from build123d import *

# Parameters (mm, degrees)
BOSS_EXTRUDE1_DEPTH = 35
SKETCH2_W           = 34.392896322
SKETCH2_H           = 15.037586703
CUT_EXTRUDE1_DEPTH  = 14
SKETCH3_R           = 2.25
CUT_EXTRUDE2_DEPTH  = 19


with BuildPart() as part:
    # Sketch1 → Boss-Extrude1 (new body)
    with BuildSketch(Plane.XY):
        with BuildLine():
            Line((-24, 0), (-14.5, 0))
            ThreePointArc((-14.5, 0), (-12.732233047, 0.732233047), (-12, 2.5))
            Line((-12, 2.5), (-12, 15.5))
            ThreePointArc((-12, 15.5), (-11.267766953, 17.267766953), (-9.5, 18))
            Line((-9.5, 18), (9.5, 18))
            ThreePointArc((9.5, 18), (11.267766953, 17.267766953), (12, 15.5))
            Line((12, 15.5), (12, 2.5))
            ThreePointArc((12, 2.5), (12.732233047, 0.732233047), (14.5, 0))
            Line((14.5, 0), (24, 0))
            Line((24, 0), (24, 2))
            Line((24, 2), (16.5, 2))
            ThreePointArc((16.5, 2), (14.732233047, 2.732233047), (14, 4.5))
            Line((14, 4.5), (14, 17.5))
            ThreePointArc((14, 17.5), (13.267766953, 19.267766953), (11.5, 20))
            Line((11.5, 20), (-11.5, 20))
            ThreePointArc((-11.5, 20), (-13.267766953, 19.267766953), (-14, 17.5))
            Line((-14, 17.5), (-14, 4.5))
            ThreePointArc((-14, 4.5), (-14.732233047, 2.732233047), (-16.5, 2))
            Line((-16.5, 2), (-24, 2))
            Line((-24, 2), (-24, 0))
        make_face()
    extrude(amount=BOSS_EXTRUDE1_DEPTH)

    # Sketch2 → Cut-Extrude1 (cut)
    with BuildSketch(Plane.XY.offset(35)):
        with Locations((0, 21.518793352)):
            Rectangle(SKETCH2_W, SKETCH2_H)
    extrude(amount=-CUT_EXTRUDE1_DEPTH, mode=Mode.SUBTRACT)

    # Sketch3 → Cut-Extrude2 (cut, symmetric)
    with BuildSketch(Plane(origin=(0, 2, 0), x_dir=(1, 0, 0), z_dir=(0, 1, 0))):
        with Locations(Location((-20.25, -5, 0), (0, 0, 90))):
            Circle(SKETCH3_R)
        with Locations(Location((-20.25, -30, 0), (0, 0, 90))):
            Circle(SKETCH3_R)
        with Locations(Location((20.25, -30, 0), (0, 0, 90))):
            Circle(SKETCH3_R)
        with Locations(Location((20.25, -5, 0), (0, 0, 90))):
            Circle(SKETCH3_R)
        with Locations(Location((0, -8, 0), (0, 0, 90))):
            Circle(SKETCH3_R)
        with Locations(Location((0, -16, 0), (0, 0, 90))):
            Circle(SKETCH3_R)
    extrude(amount=CUT_EXTRUDE2_DEPTH, both=True, mode=Mode.SUBTRACT)


solid = part.part
Design review of the part built by this model. Coordinates are the model's own, in mm. A direction names the side the tool comes from. Give positions to 0.01 mm unless a question says otherwise; leave off trailing zeros. Write each loop counter-clockwise with the first axis right and the second up, starting at its lowest first coordinate (ties: lowest second). Pieces come first, ordered by that corner, then holes. Notation, with made-up numbers: M -14,44.25 L -3,44.25 A35 cw -3,77.25 Z; hole C 16,-9.5 d5. An arc over 180 degrees is marked long. Answer as a JSON object with one key per item and string values. Group by question number.
1) We need section B-B (y = 11.5). Give the boundary of the cut face in (x, z).
2) We need section A-A (z = 16). Give the boundary of the cut face in (x, y), and give its area (3 significant figures).
3) Clearance check with flat-ended pins moving along their axes: pin 1 Ø5 at (x, y) = (18, 6.5) entering from +Z; pin 2 Ø5 at (x, z) = (20.25, 30) entering from +Y; pin 3 Ø10 at (y, z) = (11, 24) entering from +X; pin 4 Ø8 at (x, z) = (9.5, 31.5) entering from +Y. State where each tip first meets the part, or that it passes through.
4) Tool access review of faces 5 (the face through (-20, 2, 17)), 6 (the face through (-12.752, 0.713, 17.255)), 7 (the face through (-19, 0, 17)), 8 (the face through (-0.1, 18.2, 0)), 9 (the face through (-0.2, 18.4, 21)): name each direction out of +Z, -Z, +X, -X, +Y, -Y from which nothing blocks a thin tool from reaching the whole face with its end or side.
5) We need section D-D (x = 0). Give the boundary of the cut face in (y, z), and give its area (3 significant figures).
6) For line 1 along Z through (x, y) = (20.25, 1.65); line 2 along X through (y, z) = (1.2, 30); line 3 along X through (y, z) = (15.75, 19.5), list the stretches that pass through material, from the lowest coordinate up.
7) Mouldability with a two-part tool opening along Z and no side actions: class faces 1 (the face through (-18, 1, 5)), 2 (the face through (-0.676, 19.014, 13.854)), 3 (the face through (-24, 1, 17)), 4 (the face through (14, 3, 35)) as released by +Z, released by -Z, zero draft, split by the parting line, or undercut.
8) We need section C-C (z = 5). Give the boundary of the cut face in (x, y).
Answer key:
{
 "1": {"outline": "M -14,0 L -12,0 L -12,35 L -14,35 Z; M 12,0 L 14,0 L 14,35 L 12,35 Z"},
 "2": {"outline": "M -24,0 L -14.5,0 A2.5 ccw -12,2.5 L -12,15.5 A2.5 cw -9.5,18 L -2.25,18 L -2.25,20 L -11.5,20 A2.5 ccw -14,17.5 L -14,4.5 A2.5 cw -16.5,2 L -24,2 Z; M 2.25,18 L 9.5,18 A2.5 cw 12,15.5 L 12,2.5 A2.5 ccw 14.5,0 L 24,0 L 24,2 L 16.5,2 A2.5 cw 14,4.5 L 14,17.5 A2.5 ccw 11.5,20 L 2.25,20 Z", "area": "159 mm²"},
 "3": {"pin 1": "passes through", "pin 2": "stops at y = 2", "pin 3": "stops at x = 14", "pin 4": "stops at y = 14"},
 "4": {"face 5": "+Z, -Z, -X, +Y", "face 6": "+Z, -Z, -Y", "face 7": "+Z, -Z, +X, -X, -Y", "face 8": "-Z, +X, -X, +Y, -Y", "face 9": "+Z, +X, -X, +Y"},
 "5": {"outline": "M 18,0 L 20,0 L 20,5.75 L 18,5.75 Z; M 18,10.25 L 20,10.25 L 20,13.75 L 18,13.75 Z; M 18,18.25 L 20,18.25 L 20,21 L 18,21 Z", "area": "24.0 mm²"},
 "6": {"line 1": "z = 0 to 2.75, 7.25 to 27.75, 32.25 to 35", "line 2": "x = -24 to -22.5, -18 to -12.36, 12.36 to 18, 22.5 to 24", "line 3": "x = -14 to -11.99, 11.99 to 14"},
 "7": {"face 1": "undercut", "face 2": "undercut", "face 3": "zero draft", "face 4": "released by +Z"},
 "8": {"outline": "M -24,0 L -22.5,0 L -22.5,2 L -24,2 Z; M -18,0 L -14.5,0 A2.5 ccw -12,2.5 L -12,15.5 A2.5 cw -9.5,18 L 9.5,18 A2.5 cw 12,15.5 L 12,2.5 A2.5 ccw 14.5,0 L 18,0 L 18,2 L 16.5,2 A2.5 cw 14,4.5 L 14,17.5 A2.5 ccw 11.5,20 L -11.5,20 A2.5 ccw -14,17.5 L -14,4.5 A2.5 cw -16.5,2 L -18,2 Z; M 22.5,0 L 24,0 L 24,2 L 22.5,2 Z"}
}
